```python
from build123d import *

# Parameters (mm, degrees)
BASE_BLOCK_DEPTH        = 50
UPRIGHT_BODY_DEPTH      = 30
SADDLE_FLANGE_DEPTH     = 10
SIDE_BOSS_1_DEPTH       = 10
SIDE_BOSS_2_DEPTH       = 10
MOUNTING_LUG_1_SKETCH_R = 8
MOUNTING_LUG_1_DEPTH    = 10
LUG_1_BOSS_SKETCH_W     = 40
LUG_1_BOSS_SKETCH_H     = 10
LUG_1_BOSS_DEPTH        = 5
LUG_1_FILLET_R5_R       = 5
MOUNTING_LUG_2_SKETCH_R = 8
MOUNTING_LUG_2_DEPTH    = 10
LUG_2_BOSS_SKETCH_W     = 40
LUG_2_BOSS_SKETCH_H     = 10
LUG_2_BOSS_DEPTH        = 5
LUG_2_FILLET_R5_R       = 5
SIDE_RIB_DEPTH          = 50
RIB_RELIEF_CUT_DEPTH    = 15


with BuildPart() as part:
    # Base Profile Sketch → Base Block (new body)
    with BuildSketch(Plane.XY):
        with BuildLine():
            Line((-40, 0), (-30, 0))
            ThreePointArc((-30, 0), (0, 30), (30, 0))
            Line((30, 0), (40, 0))
            ThreePointArc((40, 0), (0, 40), (-40, 0))
        make_face()
    extrude(amount=BASE_BLOCK_DEPTH)



with BuildPart() as body_2:
    # Upright Profile Sketch → Upright Body (new body)
    with BuildSketch(Plane.XY.offset(50)):
        with BuildLine():
            Line((-25, 100), (-15, 100))
            ThreePointArc((-15, 100), (0, 85), (15, 100))
            Line((15, 100), (25, 100))
            ThreePointArc((25, 100), (0, 75), (-25, 100))
        make_face()
    extrude(amount=-UPRIGHT_BODY_DEPTH)



with BuildPart() as body_3:
    # Saddle Flange Sketch → Saddle Flange (new body)
    with BuildSketch(Plane.XY.offset(50)):
        with BuildLine():
            Line((-25, 100), (-39.529411765, 6.117647059))
            ThreePointArc((-39.529411765, 6.117647059), (0, 40), (39.529411765, 6.117647059))
            Line((39.529411765, 6.117647059), (25, 100))
            ThreePointArc((25, 100), (0, 75), (-25, 100))
        make_face()
    extrude(amount=SADDLE_FLANGE_DEPTH)


with BuildPart() as body_2_1:
    add(body_2.part)

    add(body_3.part)  # Side Boss 1 merges body 3
    # Side Boss 1 Sketch → Side Boss 1 (add)
    with BuildSketch(Plane.XY.offset(50)):
        with BuildLine():
            Line((-15, 100), (-25, 100))
            ThreePointArc((-25, 100), (0, 75), (25, 100))
            Line((25, 100), (15, 100))
            ThreePointArc((15, 100), (0, 85), (-15, 100))
        make_face()
    extrude(amount=SIDE_BOSS_1_DEPTH)


with BuildPart() as part_1:
    add(part.part)

    add(body_2_1.part)  # Side Boss 2 merges body 2
    # Side Boss 2 Sketch → Side Boss 2 (add)
    with BuildSketch(Plane.XY.offset(50)):
        with BuildLine():
            Line((30, 0), (40, 0))
            ThreePointArc((40, 0), (0, 40), (-40, 0))
            Line((-40, 0), (-30, 0))
            ThreePointArc((-30, 0), (0, 30), (30, 0))
        make_face()
    extrude(amount=SIDE_BOSS_2_DEPTH)



with BuildPart() as body_2_2:
    # Mounting Lug 1 Sketch → Mounting Lug 1 (new body)
    with BuildSketch(Plane.XZ):
        with BuildLine():
            Line((-60, 50), (-40, 50))
            Line((-40, 50), (-40, 10))
            Line((-40, 10), (-60, 10))
            ThreePointArc((-60, 10), (-80, 30), (-60, 50))
        make_face()
        with Locations(Location((-60, 30, 0), (0, 0, 270))):
            Circle(MOUNTING_LUG_1_SKETCH_R, mode=Mode.SUBTRACT)
    extrude(amount=-MOUNTING_LUG_1_DEPTH)


with BuildPart() as part_2:
    add(part_1.part)

    add(body_2_2.part)  # Lug 1 Boss merges body 2 2
    # Lug 1 Boss Sketch → Lug 1 Boss (add)
    with BuildSketch(Plane(origin=(-40, 0, 0), x_dir=(0, 0, -1), z_dir=(1, 0, 0))):
        with Locations((-30, 5)):
            Rectangle(LUG_1_BOSS_SKETCH_W, LUG_1_BOSS_SKETCH_H)
    extrude(amount=LUG_1_BOSS_DEPTH)

    # Lug 1 Fillet R5
    lug_1_fillet_r5_edges = [part_2.edges().sort_by_distance(p)[0] for p in [
        (-39.228991597, 8.058823529, 50),
        (-39.681187851, 5.040171699, 10),
        (-39.88217942, 3.067859955, 50),
    ]]
    fillet(lug_1_fillet_r5_edges, radius=LUG_1_FILLET_R5_R)



with BuildPart() as body_2_3:
    # Mounting Lug 2 Sketch → Mounting Lug 2 (new body)
    with BuildSketch(Plane.XZ):
        with BuildLine():
            Line((60, 50), (40, 50))
            Line((40, 50), (40, 10))
            Line((40, 10), (60, 10))
            ThreePointArc((60, 10), (80, 30), (60, 50))
        make_face()
        with Locations(Location((60, 30, 0), (0, 0, 270))):
            Circle(MOUNTING_LUG_2_SKETCH_R, mode=Mode.SUBTRACT)
    extrude(amount=-MOUNTING_LUG_2_DEPTH)


with BuildPart() as part_3:
    add(part_2.part)

    add(body_2_3.part)  # Lug 2 Boss merges body 2 3
    # Lug 2 Boss Sketch → Lug 2 Boss (add)
    with BuildSketch(Plane.ZY.offset(-40)):
        with Locations((30, 5)):
            Rectangle(LUG_2_BOSS_SKETCH_W, LUG_2_BOSS_SKETCH_H)
    extrude(amount=LUG_2_BOSS_DEPTH)

    # Lug 2 Fillet R5
    lug_2_fillet_r5_edges = [part_3.edges().sort_by_distance(p)[0] for p in [
        (39.681187851, 5.040171699, 10),
        (39.88217942, 3.067859955, 50),
        (39.228991597, 8.058823529, 50),
    ]]
    fillet(lug_2_fillet_r5_edges, radius=LUG_2_FILLET_R5_R)

    # Side Rib Sketch → Side Rib (add)
    with BuildSketch(Plane(origin=(0, 0, 50), x_dir=(-1, 0, 0), z_dir=(0, 0, -1))):
        with BuildLine():
            Line((-5, 75.505102572), (-5, 39.686269666))
            ThreePointArc((-5, 39.686269666), (0, 40), (5, 39.686269666))
            Line((5, 39.686269666), (5, 75.505102572))
            ThreePointArc((5, 75.505102572), (0, 75), (-5, 75.505102572))
        make_face()
    extrude(amount=SIDE_RIB_DEPTH)

    # Rib Relief Cut Sketch → Rib Relief Cut (cut)
    with BuildSketch(Plane.ZY.offset(5)):
        Polygon((20, 75.505102572), (0, 39.686269666), (0, 75.505102572), align=None)
    extrude(amount=-RIB_RELIEF_CUT_DEPTH, mode=Mode.SUBTRACT)


solid = part_3.part
```
Here's how the part is built. I have some questions about the finished solid (model axes, mm). A direction names the side the tool comes from. Coordinates: 2 decimals unless noted, no trailing zeros. Write each loop counter-clockwise with the first axis right and the second up, starting at its lowest first coordinate (ties: lowest second). Pieces come first, ordered by that corner, then holes. Notation, with made-up numbers: (-22, 76.5) -> (-7, 76.5) arc R32 cw to (-7, 112.5) -> close; hole circle Ø8 at (15, 51.5). An arc over 180 degrees is marked (long way). Use a Markdown table: item, result. Add a question column.
(1) Please list where these lines run through material, in increasing order: line 1 (X direction, y = 4.25, z = 30); line 2 (X direction, y = 7, z = 30); line 3 (X direction, y = 46.5, z = 24).
(2) For faces 4 (the cylindrical face through (19.516, 84.375, 35.21)), 5 (the flat face through (-52, 5, 10)), 6 (the cylindrical face through (-19.21, 84, 35.21)), 7 (the flat face through (52, 5, 10)), which set-ups out of +Z, -Z, +X, -X, +Y, -Y let a thin tool reach every point of the face, with its end or its side?
(3) We'd pull the mould along Y, two halves only. Please class faces 1 (the flat face through (-22, 56, 50)), 2 (the flat face through (49, 0, 30)), 3 (the flat face through (52, 5, 50)): +Y half, -Y half, draft (parallel to the pull), parting line (faces both ways), or undercut.
(4) I'm going to push flat-ended pins straight in: P1, Ø11, axis at x = 53, y = 5.5, coming from the -Z side; P2, Ø8, axis at x = 54.5, y = 3.5, coming from the +Z side; P3, Ø20.5, axis at x = -60.5, z = 37, coming from the +Y side. Where does each tip first touch, or does it pass through?
(5) If we section it at C-C, the plane y = 20.5: Write out the boundary of the cut face in (x, z).
(6) If we section it at B-B, the plane x = 0: Write out the boundary of the cut face in (y, z).
(7) If we section it at A-A, the plane z = 30: Write out the boundary of the cut face in (x, y), and give its area (3 significant figures).
(8) If we section it at D-D, the plane z = 16: Write out the boundary of the cut face in (x, y), and give its area (3 significant figures).
Outcome:
| question | item | result |
|---|---|---|
| 1 | line 1 | x = -80 to -68, -52 to -29.7, 29.7 to 52, 68 to 80 |
| 1 | line 2 | x = -80 to -68, -52 to -29.17, 29.17 to 52, 68 to 80 |
| 1 | line 3 | x = -5 to 5 |
| 2 | face 4 | -Z, +X |
| 2 | face 5 | -Z, -X, +Y, -Y |
| 2 | face 6 | -Z, -X |
| 2 | face 7 | -Z, +X, +Y, -Y |
| 3 | face 1 | undercut |
| 3 | face 2 | -Y half |
| 3 | face 3 | draft |
| 4 | P1 | stops at z = 10 |
| 4 | P2 | stops at z = 50 |
| 4 | P3 | stops at y = 10 |
| 5 | outline | (-37.3, 50) -> (-34.35, 50) -> (-34.35, 0) -> (-21.9, 0) -> (-21.9, 60) -> (-37.3, 60) -> close; (21.9, 0) -> (34.35, 0) -> (34.35, 50) -> (37.3, 50) -> (37.3, 60) -> (21.9, 60) -> close |
| 6 | outline | (30, 0) -> (39.69, 0) -> (75, 19.72) -> (75, 20) -> (85, 20) -> (85, 60) -> (30, 60) -> close |
| 7 | outline | (-80, 0) -> (-68, 0) -> (-68, 10) -> (-80, 10) -> close; (-52, 0) -> (-30, 0) arc R30 cw to (30, 0) -> (52, 0) -> (52, 10) -> (38.73, 10) arc R40 ccw to (5, 39.69) -> (5, 75.51) arc R25 ccw to (25, 100) -> (15, 100) arc R15 cw to (-15, 100) -> (-25, 100) arc R25 ccw to (-5, 75.51) -> (-5, 39.69) arc R40 ccw to (-38.73, 10) -> (-52, 10) -> close; (68, 0) -> (80, 0) -> (80, 10) -> (68, 10) -> close |
| 7 | area | 2,570 mm^2 |
| 8 | outline | (-74.28, 0) -> (-30, 0) arc R30 cw to (30, 0) -> (74.28, 0) -> (74.28, 10) -> (38.73, 10) arc R40 ccw to (5, 39.69) -> (5, 68.34) -> (-5, 68.34) -> (-5, 39.69) arc R40 ccw to (-38.73, 10) -> (-74.28, 10) -> close |
| 8 | area | 2,080 mm^2 |
